from build123d import *

# Parameters (mm, degrees)
SKETCH_1_R      = 1.55
SKETCH_1_R_2    = 1.9
EXTRUDE_1_DEPTH = 1.7


with BuildPart() as part:
    # 草图1 → 凸台-拉伸1 (new body)
    with BuildSketch(Plane(origin=(0, 0, 0), x_dir=(1, 0, 0), z_dir=(0, 1, 0))):
        Polygon((-55.75, -41.3), (55.75, -41.3), (55.75, 41.3), (45.35, 41.3), (45.35, 58.05), (44.35, 59.05), (25.6, 59.05), (24.6, 58.05), (24.6, 41.3), (-55.75, 41.3), align=None)
        with Locations(Location((-53, 38.5, 0), (0, 0, 270))):
            Circle(SKETCH_1_R, mode=Mode.SUBTRACT)
        with Locations(Location((53, 38.5, 0), (0, 0, 90))):
            Circle(SKETCH_1_R, mode=Mode.SUBTRACT)
        with Locations(Location((53, -38.5, 0), (0, 0, 270))):
            Circle(SKETCH_1_R, mode=Mode.SUBTRACT)
        with Locations(Location((-53, -38.5, 0), (0, 0, 90))):
            Circle(SKETCH_1_R, mode=Mode.SUBTRACT)
        with Locations(Location((29.075, 55.15, 0), (0, 0, 270))):
            Circle(SKETCH_1_R_2, mode=Mode.SUBTRACT)
        with Locations(Location((40.875, 55.15, 0), (0, 0, 90))):
            Circle(SKETCH_1_R_2, mode=Mode.SUBTRACT)
        with Locations(Location((-49.1, 17.95, 0), (0, 0, 270))):
            Circle(SKETCH_1_R, mode=Mode.SUBTRACT)
        with Locations(Location((-49.1, 6.75, 0), (0, 0, 270))):
            Circle(SKETCH_1_R, mode=Mode.SUBTRACT)
    extrude(amount=EXTRUDE_1_DEPTH)


solid = part.part
Can you work these out from the model? Positions are in its coordinate system, mm. Coordinates: 2 decimals unless noted, no trailing zeros. Order: outer loops, then holes, each group sorted by start corner. A loop starts at its lowest first (then second) coordinate and runs counter-clockwise, first axis right, second up. Notation, with made-up numbers: (-34.5, 47) - (-9.5, 47) arc R29 ccw to (-9.5, 81) - close; hole circle Ø10 at (50, -26.75). An arc over 180 degrees is marked (long way). Answer as a JSON object with one key per item and string values. Group by question number.
Q1. Imagine slicing it at B-B (z = -38.5). Please give me the cut outline in (x, y), and give its area (3 significant figures).
Q2. We'd pull the mould along Z, two halves only. Please class faces 1 (the face through (-52.534, 0.838, -37.022)), 2 (the face through (-1, 1.7, 2)): +Z half, -Z half, draft (parallel to the pull), parting line (faces both ways), or undercut.
Q3. Will these pins go through, and if not, where does the flat tip stop? P1, Ø2.5, axis at x = 53, z = 38.5, coming from the +Y side; P2, Ø0.5, axis at x = -3, y = 0.5, coming from the -Z side.
Q4. Imagine slicing it at A-A (x = -53). Please give me the cut outline in (y, z), and give its area (3 significant figures).
Q5. Imagine slicing it at C-C (z = -17.95). Please give me the cut outline in (x, y).
Q6. Imagine slicing it at D-D (y = 1.35). Give the number of separate pieces and of enclosed holes in the cut face, and give its area (3 significant figures).
Q7. I need wall thicknesses on line 1 (X direction, y = 1.1, z = -55.15) (3 decimals); line 2 (X direction, y = 0.85, z = 38.5); line 3 (X direction, y = 0.6, z = -17.95). Which ranges of each line are inside material? Lowest first, please. Write a range as from..to.
Determined:
{
 "1": {"outline": "(-55.75, 0) - (-54.55, 0) - (-54.55, 1.7) - (-55.75, 1.7) - close; (-51.45, 0) - (51.45, 0) - (51.45, 1.7) - (-51.45, 1.7) - close; (54.55, 0) - (55.75, 0) - (55.75, 1.7) - (54.55, 1.7) - close", "area": "179 mm2"},
 "2": {"face 1": "undercut", "face 2": "draft"},
 "3": {"P1": "passes through", "P2": "stops at z = -41.3"},
 "4": {"outline": "(0, -41.3) - (1.7, -41.3) - (1.7, -40.05) - (0, -40.05) - close; (0, -36.95) - (1.7, -36.95) - (1.7, 36.95) - (0, 36.95) - close; (0, 40.05) - (1.7, 40.05) - (1.7, 41.3) - (0, 41.3) - close", "area": "130 mm2"},
 "5": {"outline": "(-55.75, 0) - (-50.65, 0) - (-50.65, 1.7) - (-55.75, 1.7) - close; (-47.55, 0) - (55.75, 0) - (55.75, 1.7) - (-47.55, 1.7) - close"},
 "6": {"separate pieces": "1", "enclosed holes": "8", "area": "9,510 mm2"},
 "7": {"line 1": "x = 24.6..27.175, 30.975..38.975, 42.775..45.35", "line 2": "x = -55.75..-54.55, -51.45..51.45, 54.55..55.75", "line 3": "x = -55.75..-50.65, -47.55..55.75"}
}
